```python
from build123d import *

# Parameters (mm, degrees)
SKETCH1_R              = 12.5
BOSS_EXTRUDE1_DEPTH    = 70
M12_TAPPED_HOLE1_D     = 10.2
M12_TAPPED_HOLE1_DEPTH = 30
M12_TAPPED_HOLE1_TIP   = 3.064389157
M12_TAPPED_HOLE2_D     = 10.2
M12_TAPPED_HOLE2_DEPTH = 30
M12_TAPPED_HOLE2_TIP   = 3.064389157


with BuildPart() as part:
    # Sketch1 → Boss-Extrude1 (new body)
    with BuildSketch(Plane.XY):
        Circle(SKETCH1_R)
    extrude(amount=BOSS_EXTRUDE1_DEPTH)

    # M12 Tapped Hole1
    with Locations(Plane.XY.offset(70)):
        with Locations((0, 0)):
            Hole(M12_TAPPED_HOLE1_D / 2, depth=M12_TAPPED_HOLE1_DEPTH)
            with Locations((0, 0, -(M12_TAPPED_HOLE1_DEPTH + M12_TAPPED_HOLE1_TIP / 2))):  # 118° drill point
                Cone(0, M12_TAPPED_HOLE1_D / 2, M12_TAPPED_HOLE1_TIP, mode=Mode.SUBTRACT)

    # M12 Tapped Hole2
    with Locations(Plane(origin=(0, 0, 0), x_dir=(-1, 0, 0), z_dir=(0, 0, -1))):
        with Locations((0, 0)):
            Hole(M12_TAPPED_HOLE2_D / 2, depth=M12_TAPPED_HOLE2_DEPTH)
            with Locations((0, 0, -(M12_TAPPED_HOLE2_DEPTH + M12_TAPPED_HOLE2_TIP / 2))):  # 118° drill point
                Cone(0, M12_TAPPED_HOLE2_D / 2, M12_TAPPED_HOLE2_TIP, mode=Mode.SUBTRACT)


solid = part.part
```
Part model, mm, in its own coordinate system. A direction names the side the tool comes from. Give positions to 0.01 mm unless a question says otherwise; leave off trailing zeros. Order: outer loops, then holes, each group sorted by start corner. A loop starts at its lowest first (then second) coordinate and runs counter-clockwise, first axis right, second up. Notation, with made-up numbers: M 13.25,82 L 42.25,82 A21 cw 42.25,100 Z; hole C 82.25,-26 d5. An arc over 180 degrees is marked long. Use a Markdown table: item, result. Add a question column.
(1) Saw through at A-A, the plane z = 66. Give the cut face in (x, y), and give its area (3 significant figures).
(2) Drop flat-ended pins along their axis: P1, Ø2, axis at y = -1.5, z = 13, coming from the -X side; P2, Ø4, axis at x = 3.5, z = 28, coming from the +Y side; P3, Ø1.5, axis at y = -9.5, z = 38, coming from the +X side. Give the stop position or say it passes through.
(3) Mould opens along Y. For faces 3 (the face through (-0.2, -5.4, 70)), 4 (the face through (-2.4, -4.5, 54.8)), 5 (the face through (11.923, 3.755, 34.51)) say: +Y half, -Y half, draft (parallel to the pull), parting line (faces both ways), or undercut.
(4) Saw through at D-D, the plane y = -9. Give the cut face in (x, z), and give its area (3 significant figures).
(5) Saw through at B-B, the plane x = 10. Give the cut face in (y, z), and give its area (3 significant figures).
(6) Probe line 1 along Y through (x, z) = (0, 50); line 2 along Y through (x, z) = (2.5, 18). List the from-to ranges inside material, lowest first. Write a range as [from, to].
(7) Saw through at C-C, the plane z = 36. Give the cut face in (x, y).
(8) 3-axis set-ups, long thin cutter, end or side, ignore diameter. For faces 1 (the face through (-0.2, -5.4, 0)), 2 (the face through (2.4, -4.5, 15.2)): which of +Z, -Z, +X, -X, +Y, -Y reach the whole face in a straight line?
Answer key:
| question | item | result |
|---|---|---|
| 1 | outline | C 0,0 d25; hole C 0,0 d10.2 |
| 1 | area | 409 mm^2 |
| 2 | P1 | x = -12.49 |
| 2 | P2 | y = 12.41 |
| 2 | P3 | x = 8.93 |
| 3 | face 3 | draft |
| 3 | face 4 | undercut |
| 3 | face 5 | parting line |
| 4 | outline | M -8.67,0 L 8.67,0 L 8.67,70 L -8.67,70 Z |
| 4 | area | 1,210 mm^2 |
| 5 | outline | M -7.5,0 L 7.5,0 L 7.5,70 L -7.5,70 Z |
| 5 | area | 1,050 mm^2 |
| 6 | line 1 | [-12.5, -5.1], [5.1, 12.5] |
| 6 | line 2 | [-12.25, -4.45], [4.45, 12.25] |
| 7 | outline | C 0,0 d25 |
| 8 | face 1 | -Z, +X, -X, +Y, -Y |
| 8 | face 2 | -Z |
